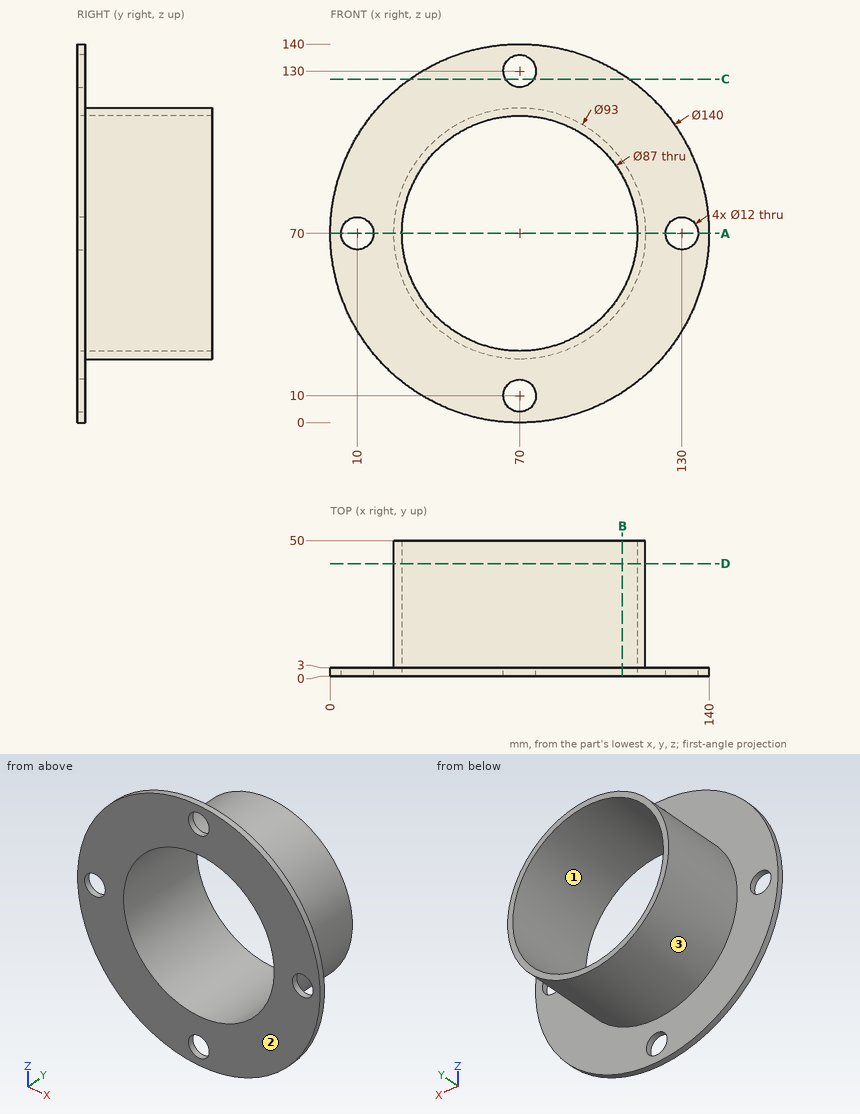
Study the drawing (mm; zero at the part's minimum x, y, z) and answer. Give positions to 0.01 mm unless a question says otherwise; leave off trailing zeros. Loops run counter-clockwise (first coordinate to the right, second up) from the corner with the lowest first, then second, coordinate; pieces in that order, holes last. Notation, with made-up numbers: (66, -29.5) - (113, -29.5) arc R34 cw to (113, 2.5) - close; hole circle Ø3 at (-6.5, 29). An arc over 180 degrees is marked (long way). Return JSON: item names as keys, results as strings. Group by question number.
1. Find section C-C (z = 127). Write down the section's boundary in (x, y), then the cut area to 3 significant figures.
2. Given pin 1 Ø12 at (x, y) = (64.5, 42) entering from -Z; pin 2 Ø4 at (y, z) = (16, 89.5) entering from -X; pin 3 Ø12 at (y, z) = (29, 49) entering from -X, each flat-ended and moving along its own axis, determine where each tip first touches the part or whether it passes through.
3. Determine the mould class of the marked faces 1, 2 and 3 for opening direction Z: pulls with the +Z half, pulls with the -Z half, needs draft (parallel to the pull), parting line crosses it, or undercut.
4. Find section A-A (z = 70). Write down the section's boundary in (x, y), then the cut area to 3 significant figures.
5. Find section B-B (x = 108). Write down the section's boundary in (y, z).
6. Find section D-D (y = 41.5). Write down the section's boundary in (x, z).
7. Straight lines are drawn through the part: line 1 (X direction, y = 1, z = 70); line 2 (X direction, y = 20, z = 70). For each, find the intervals that lie inside material, in ascending order. Write a range as [from, to].
Verdict:
{
 "1": {"outline": "(29.37, 0) - (64.8, 0) - (64.8, 3) - (29.37, 3) - close; (75.2, 0) - (110.63, 0) - (110.63, 3) - (75.2, 3) - close", "area": "213 mm^2"},
 "2": {"pin 1": "stops at z = 23.5", "pin 2": "stops at x = 26.92", "pin 3": "stops at x = 25.99"},
 "3": {"face 1": "undercut", "face 2": "needs draft", "face 3": "parting line crosses it"},
 "4": {"outline": "(0, 0) - (4, 0) - (4, 3) - (0, 3) - close; (16, 0) - (26.5, 0) - (26.5, 50) - (23.5, 50) - (23.5, 3) - (16, 3) - close; (113.5, 0) - (124, 0) - (124, 3) - (116.5, 3) - (116.5, 50) - (113.5, 50) - close; (136, 0) - (140, 0) - (140, 3) - (136, 3) - close", "area": "369 mm^2"},
 "5": {"outline": "(0, 11.21) - (3, 11.21) - (3, 43.2) - (50, 43.2) - (50, 48.83) - (0, 48.83) - close; (0, 91.17) - (50, 91.17) - (50, 96.8) - (3, 96.8) - (3, 128.79) - (0, 128.79) - close"},
 "6": {"outline": "circle Ø93 at (70, 70); hole circle Ø87 at (70, 70)"},
 "7": {"line 1": "x = [0, 4], [16, 26.5], [113.5, 124], [136, 140]", "line 2": "x = [23.5, 26.5], [113.5, 116.5]"}
}
